from build123d import *

# Parameters (mm, degrees)
BOSS_EXTRUDE1_DEPTH     = 7.75
CUT_EXTRUDE1_DEPTH      = 57.216656784
CUT_EXTRUDE1_DEPTH_BACK = 57.216656784
SKETCH3_R               = 3
SKETCH4_R               = 5.25
CUT_EXTRUDE2_DEPTH      = 5
CUT_EXTRUDE3_DEPTH      = 61.334484335
CUT_EXTRUDE3_DEPTH_BACK = 61.334484335
CHAMFER2_SIZE           = 0.5


with BuildPart() as part:
    # Sketch2 → Boss-Extrude1 (new, symmetric)
    with BuildSketch(Plane.XY):
        with BuildLine():
            Line((18, 30), (24, 30))
            Line((24, 30), (24, 12.5))
            Line((24, 12.5), (50, 12.5))
            Line((50, 12.5), (50, 4.5))
            Line((50, 4.5), (18.391574158, 4.5))
            ThreePointArc((18.391574158, 4.5), (14.050927176, 2.838262476), (11.929669724, -1.297297297))
            ThreePointArc((11.929669724, -1.297297297), (-0.649601152, -11.982404531), (-12, 0))
            ThreePointArc((-12, 0), (-3.213203436, 21.213203436), (18, 30))
        make_face()
        with BuildLine():
            Line((-2.5, 6.538348415), (-2.5, 10.5))
            Line((-2.5, 10.5), (2.5, 10.5))
            Line((2.5, 10.5), (2.5, 6.538348415))
            ThreePointArc((2.5, 6.538348415), (0, -7), (-2.5, 6.538348415))
        make_face(mode=Mode.SUBTRACT)
    extrude(amount=BOSS_EXTRUDE1_DEPTH, both=True)

    # Sketch3 → Cut-Extrude1 (cut, two sides: drawn at the far end of the back side and taken through both)
    with BuildSketch(Plane(origin=(0, 12.5, 0), x_dir=(1, 0, 0), z_dir=(0, 1, 0)).offset(-CUT_EXTRUDE1_DEPTH_BACK)):
        with Locations(Location((29, 0, 0), (0, 0, 180))):
            Circle(SKETCH3_R)
        with Locations(Location((43.5, 0, 0), (0, 0, 180))):
            Circle(SKETCH3_R)
    extrude(amount=CUT_EXTRUDE1_DEPTH + CUT_EXTRUDE1_DEPTH_BACK, mode=Mode.SUBTRACT)

    # Sketch4 → Cut-Extrude2 (cut)
    with BuildSketch(Plane.XZ.offset(-4.5)):
        with Locations((29, 0)):
            Circle(SKETCH4_R)
        with Locations((43.5, 0)):
            Circle(SKETCH4_R)
    extrude(amount=-CUT_EXTRUDE2_DEPTH, mode=Mode.SUBTRACT)

    # Sketch5 → Cut-Extrude3 (cut, two sides: drawn at the far end of the back side and taken through both)
    with BuildSketch(Plane.XY.offset(7.75).offset(-CUT_EXTRUDE3_DEPTH_BACK)):
        Polygon((24, 13.207106781), (22.585786438, 11.792893219), (23.292893219, 11.085786438), (24.707106781, 12.5), align=None)
    extrude(amount=CUT_EXTRUDE3_DEPTH + CUT_EXTRUDE3_DEPTH_BACK, mode=Mode.SUBTRACT)

    # Chamfer2
    chamfer2_edges = [part.edges().sort_by_distance(p)[0] for p in [
        (0, -7, -7.75),
        (0, -7, 7.75),
    ]]
    chamfer(chamfer2_edges, length=CHAMFER2_SIZE)


solid = part.part
Geometry check sheet. Reference: the model listing, model coordinates, mm. A direction names the side the tool comes from. Coordinates: 2 decimals unless noted, no trailing zeros. Order: outer loops, then holes, each group sorted by start corner. A loop starts at its lowest first (then second) coordinate and runs counter-clockwise, first axis right, second up. Notation, with made-up numbers: (81, 73.25) - (107, 73.25) arc R25 cw to (107, 90.25) - close; hole circle Ø6 at (-28, 85.25). An arc over 180 degrees is marked (long way). One line per item, written item: value.
(1) Sectioned sample at A-A (z = 0). Count the separate pieces of the cut face and the enclosed holes in it, and give its area (3 significant figures).
Data:
separate pieces: 3
enclosed holes: 1
area: 961 mm^2
(2) Release check for a two-part mould opening along X. For faces 4 (the face through (13, 9, 7.75)), 5 (the face through (31.3, 9.5, -2.3)), 6 (the face through (-3.445, 20.979, 0.109)) record: +X half, -X half, draft (parallel to the pull), parting line (faces both ways), or undercut.
Data:
face 4: draft
face 5: undercut
face 6: -X half
(3) Sectioned sample at C-C (x = 29). Enter the section's corners in (y, z), and give its area (3 significant figures).
Data:
outline: (4.5, -7.75) - (12.5, -7.75) - (12.5, -3) - (9.5, -3) - (9.5, -5.25) - (4.5, -5.25) - close; (4.5, 5.25) - (9.5, 5.25) - (9.5, 3) - (12.5, 3) - (12.5, 7.75) - (4.5, 7.75) - close
area: 53.5 mm^2
(4) Sectioned sample at D-D (z = -4.25). Enter the section's corners in (x, y).
Data:
outline: (-12, 0) arc R12 ccw to (11.93, -1.3) arc R6.5 cw to (18.39, 4.5) - (25.92, 4.5) - (25.92, 9.5) - (32.08, 9.5) - (32.08, 4.5) - (40.42, 4.5) - (40.42, 9.5) - (46.58, 9.5) - (46.58, 4.5) - (50, 4.5) - (50, 12.5) - (24.71, 12.5) - (23.29, 11.09) - (22.59, 11.79) - (24, 13.21) - (24, 30) - (18, 30) arc R30 ccw to start; hole (-2.5, 6.54) arc R7 ccw (long way) to (2.5, 6.54) - (2.5, 10.5) - (-2.5, 10.5) - close
(5) Sectioned sample at B-B (x = 0). Enter the section's corners in (y, z).
Data:
outline: (-12, -7.75) - (-7.5, -7.75) - (-7, -7.25) - (-7, 7.25) - (-7.5, 7.75) - (-12, 7.75) - close; (10.5, -7.75) - (24, -7.75) - (24, 7.75) - (10.5, 7.75) - close
(6) Access from +Z, -Z, +X, -X, +Y, -Y to the whole of each face (thin tool, end or side, straight path). Record for faces 1 (the face through (39.63, 6.96, 3.55)), 2 (the face through (37, 12.5, 0)), 3 (the face through (0, 10.5, 0)).
Data:
face 1: -Y
face 2: +Z, -Z, +X, +Y
face 3: +Z, -Z
(7) Depth check by flat-ended pin: pin 1 Ø8.5 at (x, z) = (27, -1) entering from -Y; pin 2 Ø4 at (x, z) = (6.5, 2) entering from +Y; pin 3 Ø8 at (x, z) = (29, 0) entering from +Y. Enter the tip coordinate at first touch or a pass-through.
Data:
pin 1: stops at y = 4.5
pin 2: stops at y = 28.46
pin 3: stops at y = 12.5
(8) Thickness scan on probe 1 along Z at (x, y) = (43.5, 11.4); probe 2 along X at (y, z) = (10.65, 0); probe 3 along Z at (x, y) = (29, 7.3). Record the ranges inside material, lowest first. Write a range as from..to.
Data:
probe 1: z = -7.75..-3, 3..7.75
probe 2: x = -10.05..26, 32..40.5, 46.5..50
probe 3: z = -7.75..-5.25, 5.25..7.75
